Here's how the part is built. I have some questions about the finished solid (model axes, mm). A direction names the side the tool comes from. Round coordinates to 2 decimals unless told otherwise and drop trailing zeros. Loops run counter-clockwise (first coordinate to the right, second up) from the corner with the lowest first, then second, coordinate; pieces in that order, holes last. Notation, with made-up numbers: (-6.5, -32.75) -> (15.5, -32.75) arc R25 cw to (15.5, -3.75) -> close; hole circle Ø6 at (-5.75, 17.25). An arc over 180 degrees is marked (long way). Use one line per item in the form item = value. Start each with the question number.
Item 1: For faces 1 (the face through (-1, -60, 15)), 2 (the face through (-493, -325, 12)), 3 (the face through (-249.44, -232.615, 20.14)), 4 (the face through (493, -325, 12)), which set-ups out of +Z, -Z, +X, -X, +Y, -Y let a thin tool reach every point of the face, with its end or its side?
Item 2: If we section it at A-A (x = 44): Write out the boundary of the cut face in (y, z).
Item 3: If I drill on L1, parallel to Y at x = 488, z = 17.5; L2, parallel to X at y = 45.5, z = 3.25, over which ranges is the centre line in solid material (lowest first)? Write a range as [from, to].
Item 4: I'm going to push flat-ended pins straight in: pin 1 Ø4 at (x, z) = (315, 17.5) entering from +Y; pin 2 Ø3 at (x, z) = (336, 20) entering from -Y; pin 3 Ø5.5 at (y, z) = (315, 17.5) entering from -X. Where does each tip first touch, or does it pass through?
```python
from build123d import *

# Parameters (mm, degrees)
SKETCH1_W                  = 1000
SKETCH1_H                  = 1000
SKETCH1_W_2                = 120
SKETCH1_H_2                = 120
BOSS_EXTRUDE1_DEPTH        = 30
SKETCH2_R                  = 15
CUT_EXTRUDE1_DEPTH         = 20
SKETCH3_W                  = 50
SKETCH3_H                  = 90
CUT_EXTRUDE2_DEPTH         = 7
CIRPATTERN1_COUNT          = 4
M4_TAPPED_HOLE1_AT_2_COUNT = 2
M4_TAPPED_HOLE1_AT_2_PITCH = 20
M4_TAPPED_HOLE1_AT_3_COUNT = 2
M4_TAPPED_HOLE1_AT_3_PITCH = 650
M4_TAPPED_HOLE1_AT_4_COUNT = 2
M4_TAPPED_HOLE1_AT_4_PITCH = 670
CIRPATTERN2_COUNT          = 4


with BuildPart() as part:
    # Sketch1 → Boss-Extrude1 (new body)
    with BuildSketch(Plane.XY):
        Rectangle(SKETCH1_W, SKETCH1_H)
        Rectangle(SKETCH1_W_2, SKETCH1_H_2, mode=Mode.SUBTRACT)
    extrude(amount=BOSS_EXTRUDE1_DEPTH)

    # Sketch2 → Cut-Extrude1 (cut)
    with BuildSketch(Plane.XY.offset(30)):
        with Locations((-247.487373415, 247.487373415)):
            Circle(SKETCH2_R)
        with Locations((247.487373415, 247.487373415)):
            Circle(SKETCH2_R)
        with Locations((247.487373415, -247.487373415)):
            Circle(SKETCH2_R)
        with Locations((-247.487373415, -247.487373415)):
            Circle(SKETCH2_R)
    extrude(amount=-CUT_EXTRUDE1_DEPTH, mode=Mode.SUBTRACT)

    # Sketch3 → Cut-Extrude2 (cut)
    with BuildSketch(Plane(origin=(0, 500, 0), x_dir=(1, 0, 0), z_dir=(0, 1, 0))):
        with Locations((-325, 20)):
            Rectangle(SKETCH3_W, SKETCH3_H)
        with Locations((325, 20)):
            Rectangle(SKETCH3_W, SKETCH3_H)
    cut_extrude2 = extrude(amount=-CUT_EXTRUDE2_DEPTH, mode=Mode.SUBTRACT)

    # CirPattern1: Cut-Extrude2 ×4 about axis
    cirpattern1_axis = Axis((0, 0, 0), (0, 0, 1))
    for i in range(1, CIRPATTERN1_COUNT):
        add(cut_extrude2.rotate(cirpattern1_axis, i * 360 / CIRPATTERN1_COUNT), mode=Mode.SUBTRACT)

    # Sketch6 → M4 Tapped Hole1 (revolve, cut)
    with BuildSketch(Plane(origin=(335, -493, 17.5), x_dir=(0, 0, -1), z_dir=(1, 0, 0))):
        Polygon((0, 0), (0, 11.091420021), (1.65, 10.1), (1.65, 0), align=None)
    m4_tapped_hole1 = revolve(axis=Axis((335, -499.35, 17.5), (0, 1, 0)), mode=Mode.SUBTRACT)

    # M4 Tapped Hole1 at 2: M4 Tapped Hole1 ×2
    with Locations(*[(-i * M4_TAPPED_HOLE1_AT_2_PITCH, 0, 0) for i in range(1, M4_TAPPED_HOLE1_AT_2_COUNT)]):
        add(m4_tapped_hole1, mode=Mode.SUBTRACT)

    # M4 Tapped Hole1 at 3: M4 Tapped Hole1 ×2
    with Locations(*[(-i * M4_TAPPED_HOLE1_AT_3_PITCH, 0, 0) for i in range(1, M4_TAPPED_HOLE1_AT_3_COUNT)]):
        add(m4_tapped_hole1, mode=Mode.SUBTRACT)

    # M4 Tapped Hole1 at 4: M4 Tapped Hole1 ×2
    with Locations(*[(-i * M4_TAPPED_HOLE1_AT_4_PITCH, 0, 0) for i in range(1, M4_TAPPED_HOLE1_AT_4_COUNT)]):
        add(m4_tapped_hole1, mode=Mode.SUBTRACT)

    # CirPattern2: M4 Tapped Hole1 ×4 about axis
    cirpattern2_axis = Axis((0, 0, 0), (0, 0, -1))
    for i in range(1, CIRPATTERN2_COUNT):
        add(m4_tapped_hole1.rotate(cirpattern2_axis, i * 360 / CIRPATTERN2_COUNT), mode=Mode.SUBTRACT)

    # CirPattern2 copy 1 sketch → CirPattern2 copy 1 (revolve, cut)
    with BuildSketch(Plane(origin=(-493, -315, 17.5), x_dir=(0, 0, -1), z_dir=(0, -1, 0))):
        Polygon((0, 0), (0, 11.091420021), (1.65, 10.1), (1.65, 0), align=None)
    revolve(axis=Axis((-499.35, -315, 17.5), (1, 0, 0)), mode=Mode.SUBTRACT)

    # CirPattern2 copy 2 sketch → CirPattern2 copy 2 (revolve, cut)
    with BuildSketch(Plane(origin=(-315, 493, 17.5), x_dir=(0, 0, -1), z_dir=(-1, 0, 0))):
        Polygon((0, 0), (0, 11.091420021), (1.65, 10.1), (1.65, 0), align=None)
    revolve(axis=Axis((-315, 499.35, 17.5), (0, -1, 0)), mode=Mode.SUBTRACT)

    # CirPattern2 copy 3 sketch → CirPattern2 copy 3 (revolve, cut)
    with BuildSketch(Plane(origin=(493, 315, 17.5), x_dir=(0, 0, -1), z_dir=(0, 1, 0))):
        Polygon((0, 0), (0, 11.091420021), (1.65, 10.1), (1.65, 0), align=None)
    revolve(axis=Axis((499.35, 315, 17.5), (-1, 0, 0)), mode=Mode.SUBTRACT)

    # CirPattern2 copy 4 sketch → CirPattern2 copy 4 (revolve, cut)
    with BuildSketch(Plane(origin=(-493, 315, 17.5), x_dir=(0, 0, -1), z_dir=(0, -1, 0))):
        Polygon((0, 0), (0, 11.091420021), (1.65, 10.1), (1.65, 0), align=None)
    revolve(axis=Axis((-499.35, 315, 17.5), (1, 0, 0)), mode=Mode.SUBTRACT)

    # CirPattern2 copy 5 sketch → CirPattern2 copy 5 (revolve, cut)
    with BuildSketch(Plane(origin=(315, 493, 17.5), x_dir=(0, 0, -1), z_dir=(-1, 0, 0))):
        Polygon((0, 0), (0, 11.091420021), (1.65, 10.1), (1.65, 0), align=None)
    revolve(axis=Axis((315, 499.35, 17.5), (0, -1, 0)), mode=Mode.SUBTRACT)

    # CirPattern2 copy 6 sketch → CirPattern2 copy 6 (revolve, cut)
    with BuildSketch(Plane(origin=(493, -315, 17.5), x_dir=(0, 0, -1), z_dir=(0, 1, 0))):
        Polygon((0, 0), (0, 11.091420021), (1.65, 10.1), (1.65, 0), align=None)
    revolve(axis=Axis((499.35, -315, 17.5), (-1, 0, 0)), mode=Mode.SUBTRACT)

    # CirPattern2 copy 7 sketch → CirPattern2 copy 7 (revolve, cut)
    with BuildSketch(Plane(origin=(-493, 335, 17.5), x_dir=(0, 0, -1), z_dir=(0, -1, 0))):
        Polygon((0, 0), (0, 11.091420021), (1.65, 10.1), (1.65, 0), align=None)
    revolve(axis=Axis((-499.35, 335, 17.5), (1, 0, 0)), mode=Mode.SUBTRACT)

    # CirPattern2 copy 8 sketch → CirPattern2 copy 8 (revolve, cut)
    with BuildSketch(Plane(origin=(335, 493, 17.5), x_dir=(0, 0, -1), z_dir=(-1, 0, 0))):
        Polygon((0, 0), (0, 11.091420021), (1.65, 10.1), (1.65, 0), align=None)
    revolve(axis=Axis((335, 499.35, 17.5), (0, -1, 0)), mode=Mode.SUBTRACT)

    # CirPattern2 copy 9 sketch → CirPattern2 copy 9 (revolve, cut)
    with BuildSketch(Plane(origin=(493, -335, 17.5), x_dir=(0, 0, -1), z_dir=(0, 1, 0))):
        Polygon((0, 0), (0, 11.091420021), (1.65, 10.1), (1.65, 0), align=None)
    revolve(axis=Axis((499.35, -335, 17.5), (-1, 0, 0)), mode=Mode.SUBTRACT)


solid = part.part
```
Values found:
q1.face_1 = +Z, -Z
q1.face_2 = -Z, -X
q1.face_3 = +Z
q1.face_4 = -Z, +X
q2.outline = (-500, 0) -> (-60, 0) -> (-60, 30) -> (-500, 30) -> close; (60, 0) -> (500, 0) -> (500, 30) -> (60, 30) -> close
q3.L1 = [-500, -336.65], [-333.35, -316.65], [-313.35, 313.35], [316.65, 333.35], [336.65, 500]
q3.L2 = [-500, -60], [60, 500]
q4.pin_1 = 493
q4.pin_2 = -493
q4.pin_3 = -493
